Can you work these out from the drawing? Everything is in mm from the part's minimum corner. Coordinates: 2 decimals unless noted, no trailing zeros. Order: outer loops, then holes, each group sorted by start corner. A loop starts at its lowest first (then second) coordinate and runs counter-clockwise, first axis right, second up. Notation, with made-up numbers: (38, 5.25) - (50, 5.25) arc R29 cw to (50, 33.25) - close; hole circle Ø2 at (-9.75, 89.25). An arc over 180 degrees is marked (long way). Answer as CSV lines item,"result". Start each with the question number.
Q1. For pin 1 Ø2 at (x, z) = (99, 7.5) entering from -Y; pin 2 Ø4 at (x, y) = (97.5, 51) entering from +Z, each with a flat end and sliding along its axis, tell me the tip position at first contact or that it passes through.
Q2. Thinking about a two-plate mould opening in X: for the marked faces 1 and 2, which applies, released by +X, released by -X, zero draft, split by the parting line, or undercut?
Q3. Suppose I cut it at A-A (y = 9). Please give me the cut outline in (x, z).
Q4. I need wall thicknesses on line 1 (Y direction, x = 152.5, z = 6); line 2 (X direction, y = 52, z = 2.5); line 3 (Y direction, x = 30, z = 4). Which ranges of each line are inside material? Lowest first, please.
Q5. Suppose I cut it at D-D (z = 5.5). Please give me the cut outline in (x, y), then the cut area to 3 significant figures.
Q6. Suppose I cut it at C-C (x = 30). Please give me the cut outline in (y, z), then the cut area to 3 significant figures.
Q7. Suppose I cut it at B-B (x = 97.5). Please give me the cut outline in (y, z), then the cut area to 3 significant figures.
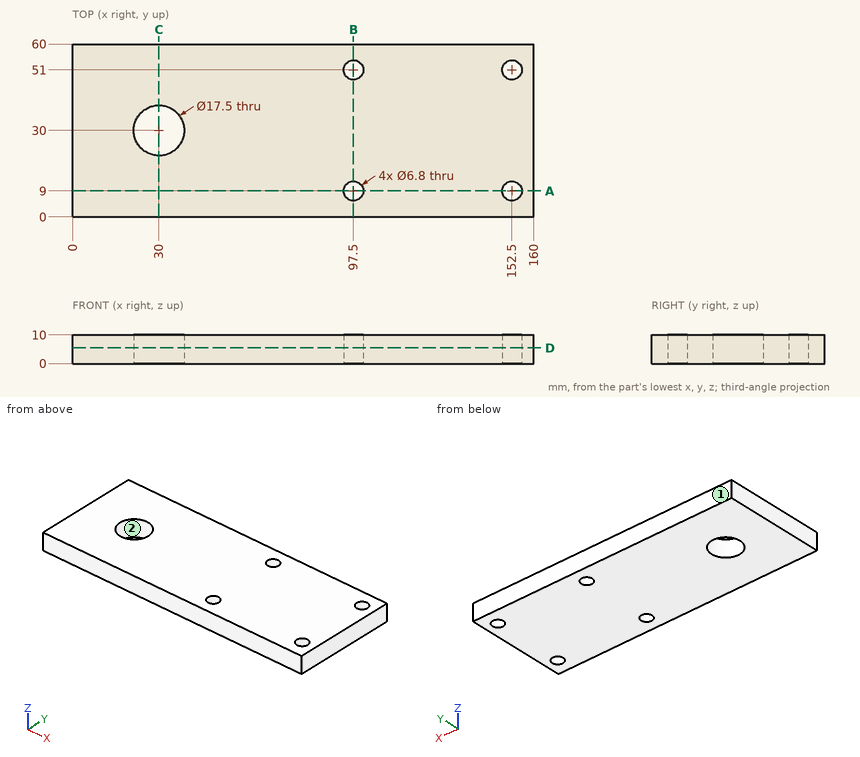
Here are the results:
1,pin 1,"stops at y = 0"
1,pin 2,"passes through"
2,face 1,"zero draft"
2,face 2,"undercut"
3,outline,"(0, 0) - (94.1, 0) - (94.1, 10) - (0, 10) - close; (100.9, 0) - (149.1, 0) - (149.1, 10) - (100.9, 10) - close; (155.9, 0) - (160, 0) - (160, 10) - (155.9, 10) - close"
4,line 1,"y = 0 to 5.6, 12.4 to 47.6, 54.4 to 60"
4,line 2,"x = 0 to 94.25, 100.75 to 149.25, 155.75 to 160"
4,line 3,"y = 0 to 21.25, 38.75 to 60"
5,outline,"(0, 0) - (160, 0) - (160, 60) - (0, 60) - close; hole circle Ø17.5 at (30, 30); hole circle Ø6.8 at (97.5, 9); hole circle Ø6.8 at (97.5, 51); hole circle Ø6.8 at (152.5, 9); hole circle Ø6.8 at (152.5, 51)"
5,area,"9,210 mm²"
6,outline,"(0, 0) - (21.25, 0) - (21.25, 10) - (0, 10) - close; (38.75, 0) - (60, 0) - (60, 10) - (38.75, 10) - close"
6,area,"425 mm²"
7,outline,"(0, 0) - (5.6, 0) - (5.6, 10) - (0, 10) - close; (12.4, 0) - (47.6, 0) - (47.6, 10) - (12.4, 10) - close; (54.4, 0) - (60, 0) - (60, 10) - (54.4, 10) - close"
7,area,"464 mm²"
